Verification items for the finished model (mm, model axes). Face numbers are marked on the shaded views. A direction names the side the tool comes from. Round coordinates to 2 decimals unless told otherwise and drop trailing zeros. Order: outer loops, then holes, each group sorted by start corner. A loop starts at its lowest first (then second) coordinate and runs counter-clockwise, first axis right, second up. Notation, with made-up numbers: (18.5, 22) -> (64.5, 22) arc R10 ccw to (64.5, 34) -> close; hole circle Ø4 at (35.25, -6.5). An arc over 180 degrees is marked (long way). Put each result on its own line as item: value.
from build123d import *

# Parameters (mm, degrees)
SKETCH1_R                                          = 5
BOSS_EXTRUDE1_DEPTH                                = 18
HOLE_WIZARD_SOCKET_HEAD_CAP_SCREW_TYPE_D           = 4.5
HOLE_WIZARD_SOCKET_HEAD_CAP_SCREW_TYPE_CBORE_D     = 8
HOLE_WIZARD_SOCKET_HEAD_CAP_SCREW_TYPE_CBORE_DEPTH = 4.6
CHAMFER1_SIZE                                      = 0.5


with BuildPart() as part:
    # Sketch1 → Boss-Extrude1 (new body)
    with BuildSketch(Plane(origin=(0, 0, 0), x_dir=(1, 0, 0), z_dir=(0, 1, 0))):
        with Locations(Location((0, 0, 0), (0, 0, 270))):
            Circle(SKETCH1_R)
    extrude(amount=BOSS_EXTRUDE1_DEPTH)

    # Hole wizard: socket head cap screw, type 1 (through all)
    with Locations(Plane(origin=(0, 18, 0), x_dir=(1, 0, 0), z_dir=(0, 1, 0))):
        with Locations((0, 0)):
            CounterBoreHole(HOLE_WIZARD_SOCKET_HEAD_CAP_SCREW_TYPE_D / 2, HOLE_WIZARD_SOCKET_HEAD_CAP_SCREW_TYPE_CBORE_D / 2, HOLE_WIZARD_SOCKET_HEAD_CAP_SCREW_TYPE_CBORE_DEPTH)

    # Chamfer1
    chamfer1_edges = [part.edges().sort_by_distance(p)[0] for p in [
        (0, 18, -5),
    ]]
    chamfer(chamfer1_edges, length=CHAMFER1_SIZE)


solid = part.part
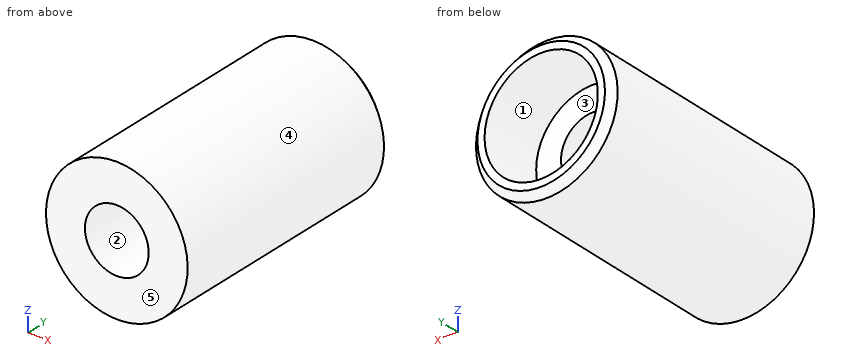
Item 1: Section check A-A on x = 0. Record the boundary of the cut face in (y, z).
Check sheet entries:
outline: (0, -5) -> (17.5, -5) -> (18, -4.5) -> (18, -4) -> (13.4, -4) -> (13.4, -2.25) -> (0, -2.25) -> close; (0, 2.25) -> (13.4, 2.25) -> (13.4, 4) -> (18, 4) -> (18, 4.5) -> (17.5, 5) -> (0, 5) -> close
Item 2: Section check C-C on y = 9. Record the boundary of the cut face in (x, z), then the cut area to 3 significant figures.
Check sheet entries:
outline: circle Ø10 at (0, 0); hole circle Ø4.5 at (0, 0)
area: 62.6 mm^2
Item 3: Gauge pin test, flat ends, axial feed: pin 1 Ø2 at (x, y) = (3.5, 12) entering from +Z; pin 2 Ø1.5 at (x, y) = (1.5, 6) entering from -Z; pin 3 Ø1 at (x, z) = (-1.5, -2) entering from +Y. Record the tip position at first contact, or that the pin passes through.
Check sheet entries:
pin 1: stops at z = 4.33
pin 2: stops at z = -4.94
pin 3: stops at y = 13.4
Item 4: Release check for a two-part mould opening along X. For the marked faces 3, 4 and 5 record: +X half, -X half, draft (parallel to the pull), parting line (faces both ways), or undercut.
Check sheet entries:
face 3: undercut
face 4: parting line
face 5: draft
Item 5: Tool access check on the marked faces 1 and 2. Record the directions out of +Z, -Z, +X, -X, +Y, -Y that give a thin tool (end or side, any length) a straight path to the whole face; none if there is none.
Check sheet entries:
face 1: +Y
face 2: +Y, -Y
Item 6: Material ranges on L1, parallel to X at y = 13.25, z = -1; L2, parallel to Z at x = 0.75, y = 13.5; L3, parallel to Y at x = -2.5, z = -2.5, recorded low to high. Write a range as [from, to].
Check sheet entries:
L1: x = [-4.9, -2.02], [2.02, 4.9]
L2: z = [-4.94, -3.93], [3.93, 4.94]
L3: y = [0, 13.4]
Item 7: Section check B-B on z = 0. Record the boundary of the cut face in (x, y), then the cut area to 4 significant figures.
Check sheet entries:
outline: (-5, 0) -> (-2.25, 0) -> (-2.25, 13.4) -> (-4, 13.4) -> (-4, 18) -> (-4.5, 18) -> (-5, 17.5) -> close; (2.25, 0) -> (5, 0) -> (5, 17.5) -> (4.5, 18) -> (4, 18) -> (4, 13.4) -> (2.25, 13.4) -> close
area: 82.65 mm^2
